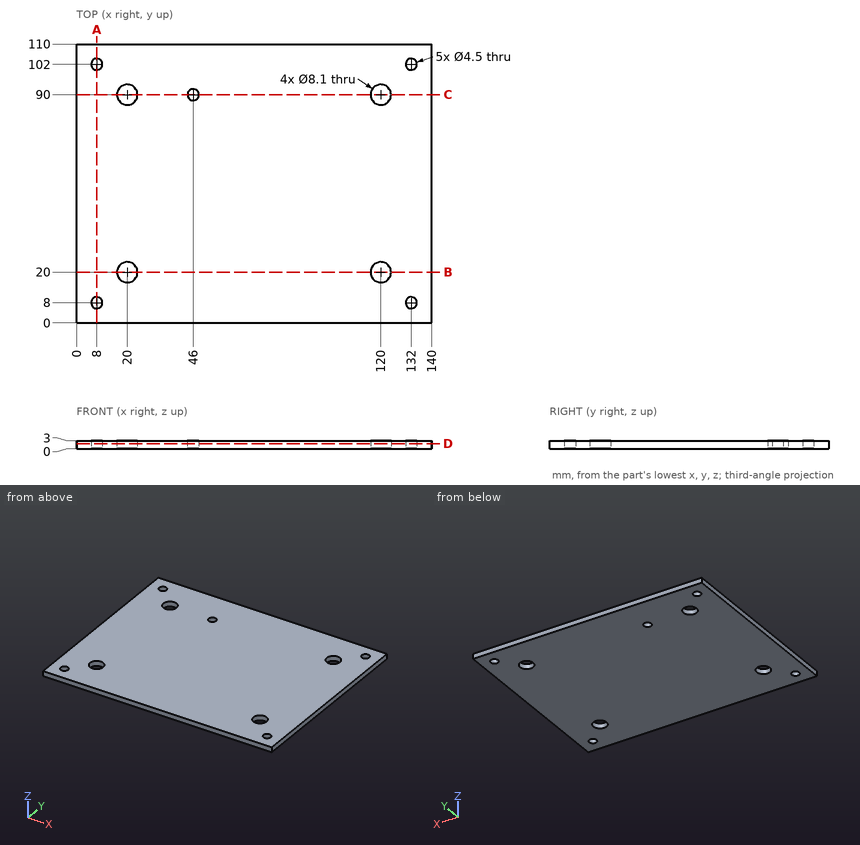
Answer from the drawing. Dimensions are ordinates in mm from the lowest x, y and z of the part. Give positions to 0.01 mm unless a question says otherwise; leave off trailing zeros. Loops run counter-clockwise (first coordinate to the right, second up) from the corner with the lowest first, then second, coordinate; pieces in that order, holes last. Notation, with made-up numbers: (25, -40) - (84, -40) arc R16 cw to (84, -11) - close; hole circle Ø8 at (-8.5, 39). An arc over 180 degrees is marked (long way). Answer as a JSON object with one key per item and string values.
1. A cutting plane is placed at D-D (z = 1.9). Give the number of separate pieces and of enclosed holes in the cut face, then the cut area to 3 significant figures.
Determined:
{"separate pieces": "1", "enclosed holes": "9", "area": "15,100 mm²"}
2. A cutting plane is placed at B-B (y = 20). Write down the section's boundary in (x, z), then the cut area to 3 significant figures.
Determined:
{"outline": "(0, 0) - (15.95, 0) - (15.95, 3) - (0, 3) - close; (24.05, 0) - (115.95, 0) - (115.95, 3) - (24.05, 3) - close; (124.05, 0) - (140, 0) - (140, 3) - (124.05, 3) - close", "area": "371 mm²"}
3. A cutting plane is placed at A-A (x = 8). Write down the section's boundary in (y, z).
Determined:
{"outline": "(0, 0) - (5.75, 0) - (5.75, 3) - (0, 3) - close; (10.25, 0) - (99.75, 0) - (99.75, 3) - (10.25, 3) - close; (104.25, 0) - (110, 0) - (110, 3) - (104.25, 3) - close"}
4. A cutting plane is placed at C-C (y = 90). Write down the section's boundary in (x, z).
Determined:
{"outline": "(0, 0) - (15.95, 0) - (15.95, 3) - (0, 3) - close; (24.05, 0) - (43.75, 0) - (43.75, 3) - (24.05, 3) - close; (48.25, 0) - (115.95, 0) - (115.95, 3) - (48.25, 3) - close; (124.05, 0) - (140, 0) - (140, 3) - (124.05, 3) - close"}
5. A flat-ended cylindrical pin translates along its axis: pin 1 Ø3.5 at (x, y) = (132, 8) entering from +Z. Find the tip coordinate at first contact, or state that the pin passes through.
Determined:
{"pin 1": "through"}
6. Find the intervals of material crossed by L1, parallel to Y at x = 20, z = 1.5; L2, parallel to Y at x = 132, z = 0.9; L3, parallel to X at y = 93, z = 1.5, in increasing order. Write a range as [from, to].
Determined:
{"L1": "[0, 15.95], [24.05, 85.95], [94.05, 110]", "L2": "[0, 5.75], [10.25, 99.75], [104.25, 110]", "L3": "[0, 17.28], [22.72, 117.28], [122.72, 140]"}
